from build123d import *

# Parameters (mm, degrees)
SKETCH1_R           = 12.5
BOSS_EXTRUDE1_DEPTH = 20
SKETCH2_R           = 10
BOSS_EXTRUDE2_DEPTH = 75
SKETCH3_R           = 7
BOSS_EXTRUDE3_DEPTH = 10


with BuildPart() as part:
    # Sketch1 → Boss-Extrude1 (new body)
    with BuildSketch(Plane(origin=(0, 0, 0), x_dir=(1, 0, 0), z_dir=(0, 1, 0))):
        with Locations(Location((0, 0, 0), (0, 0, 270))):
            Circle(SKETCH1_R)
    extrude(amount=BOSS_EXTRUDE1_DEPTH)

    # Sketch2 → Boss-Extrude2 (add)
    with BuildSketch(Plane(origin=(0, 20, 0), x_dir=(1, 0, 0), z_dir=(0, 1, 0))):
        with Locations(Location((0, 0, 0), (0, 0, 270))):
            Circle(SKETCH2_R)
    extrude(amount=BOSS_EXTRUDE2_DEPTH)

    # Sketch3 → Boss-Extrude3 (add)
    with BuildSketch(Plane(origin=(0, 95, 0), x_dir=(1, 0, 0), z_dir=(0, 1, 0))):
        with Locations(Location((0, 0, 0), (0, 0, 270))):
            Circle(SKETCH3_R)
    extrude(amount=BOSS_EXTRUDE3_DEPTH)


solid = part.part
Work out the finished part from the listing and answer in its coordinate system (mm). Give positions to 0.01 mm unless a question says otherwise; leave off trailing zeros. Loops run counter-clockwise (first coordinate to the right, second up) from the corner with the lowest first, then second, coordinate; pieces in that order, holes last. Notation, with made-up numbers: (84, 45) -> (99, 45) arc R12 cw to (99, 68) -> close; hole circle Ø4 at (59.25, -23). An arc over 180 degrees is marked (long way). Use a Markdown table: item, result. Add a question column.
1. Flat-ended cylindrical pins translate along their axes: pin 1 Ø10 at (x, y) = (-7.5, 52.5) entering from +Z; pin 2 Ø10 at (x, y) = (0, 40) entering from +Z; pin 3 Ø4 at (y, z) = (14, -5) entering from +X. Find the tip coordinate at first contact, or state that the pin passes through.
2. Determine the mould class of faces 1 (the flat face through (0, 105, 0)), 2 (the cylindrical face through (3.755, 9.86, 11.923)), 3 (the flat face through (0, 0, 0)) for opening direction Y: released by +Y, released by -Y, zero draft, split by the parting line, or undercut.
3. Section A-A on z = 0 is taken. Determine the outline of the cut face in (x, y), and give its area (3 significant figures).
4. Section C-C on y = 8.5 is taken. Determine the outline of the cut face in (x, z).
5. Find the intervals of material crossed by probe 1 along Y at (x, z) = (-7.5, 4); probe 2 along Z at (x, y) = (0.25, 54); probe 3 along Y at (x, z) = (11, -4.25), in increasing order.
6. Section D-D on y = 48 is taken. Determine the outline of the cut face in (x, z), and give its area (3 significant figures).
7. Section B-B on x = 0 is taken. Determine the outline of the cut face in (y, z).
Results below:
| question | item | result |
|---|---|---|
| 1 | pin 1 | stops at z = 9.68 |
| 1 | pin 2 | stops at z = 10 |
| 1 | pin 3 | stops at x = 12.13 |
| 2 | face 1 | released by +Y |
| 2 | face 2 | zero draft |
| 2 | face 3 | released by -Y |
| 3 | outline | (-12.5, 0) -> (12.5, 0) -> (12.5, 20) -> (10, 20) -> (10, 95) -> (7, 95) -> (7, 105) -> (-7, 105) -> (-7, 95) -> (-10, 95) -> (-10, 20) -> (-12.5, 20) -> close |
| 3 | area | 2,140 mm^2 |
| 4 | outline | circle Ø25 at (0, 0) |
| 5 | probe 1 | y = 0 to 95 |
| 5 | probe 2 | z = -10 to 10 |
| 5 | probe 3 | y = 0 to 20 |
| 6 | outline | circle Ø20 at (0, 0) |
| 6 | area | 314 mm^2 |
| 7 | outline | (0, -12.5) -> (20, -12.5) -> (20, -10) -> (95, -10) -> (95, -7) -> (105, -7) -> (105, 7) -> (95, 7) -> (95, 10) -> (20, 10) -> (20, 12.5) -> (0, 12.5) -> close |
